Can you work these out from the model? Positions are in its coordinate system, mm. Coordinates: 2 decimals unless noted, no trailing zeros. Loops run counter-clockwise (first coordinate to the right, second up) from the corner with the lowest first, then second, coordinate; pieces in that order, holes last.
```python
from build123d import *

# Parameters (mm, degrees)
G1_1_4_TAPPED_HOLE1_D = 39.25
CHAMFER1_SIZE         = 1


with BuildPart() as part:
    # Sketch1 → Revolve1 (revolve)
    with BuildSketch(Plane(origin=(0, 0, 0), x_dir=(0, 0, -1), z_dir=(1, 0, 0)), mode=Mode.PRIVATE) as revolve1_sk:
        Polygon((0, 0), (0, 25), (-10, 25), (-10, 30), (-20, 30), (-20, 0), align=None)
    revolve(revolve1_sk.sketch.rotate(Axis((0, 0, 20), (0, 0, -1)), 90), axis=Axis((0, 0, 20), (0, 0, -1)))

    # G1-1/4 Tapped Hole1 (through all)
    with Locations(Plane.XY.offset(20)):
        with Locations((0, 0)):
            Hole(G1_1_4_TAPPED_HOLE1_D / 2)

    # Chamfer1
    chamfer1_edges = [part.edges().sort_by_distance(p)[0] for p in [
        (-30, 0, 20),
    ]]
    chamfer(chamfer1_edges, length=CHAMFER1_SIZE)


solid = part.part
```
(1) I want a section at A-A on x = 0. Write out the boundary of the cut face in (y, z) (3 decimals), then the cut area to 3 significant figures.
Check values:
outline: (-30, 10) - (-25, 10) - (-25, 0) - (-19.625, 0) - (-19.625, 20) - (-29, 20) - (-30, 19) - close; (19.625, 0) - (25, 0) - (25, 10) - (30, 10) - (30, 19) - (29, 20) - (19.625, 20) - close
area: 314 mm2
(2) If we mould it in two halves opening along X, with no side actions, what happens to faces 1 (the cylindrical face through (23.846, -7.509, 5.07)), 2 (the flat face through (7, -25, 10)), 3 (the cylindrical face through (19.606, 0.863, 9.86))? For each: released by +X, released by -X, zero draft, split by the parting line, or undercut.
Check values:
face 1: split by the parting line
face 2: zero draft
face 3: undercut
(3) I want a section at C-C on z = 6.75. Write out the boundary of the cut face in (x, y) (3 decimals), then the cut area to 3 significant figures.
Check values:
outline: circle Ø50 at (0, 0); hole circle Ø39.25 at (0, 0)
area: 754 mm2
(4) I'm going to push flat-ended pins straight in: pin 1 (10 mm diameter, centred on x = -13.5, z = 10.5, fed in from +Y); pin 2 (3 mm diameter, centred on y = 10.5, z = 6, fed in from -X); pin 3 (5 mm diameter, centred on x = 0, z = 13, fed in from -Y); pin 4 (23.5 mm diameter, centred on x = 0, y = 0, fed in from -Z). Where does each tip first touch, or does it pass through?
Check values:
pin 1: stops at y = 28.77
pin 2: stops at x = -23.32
pin 3: stops at y = -30
pin 4: passes through
(5) If I drill on probe 1 along Y at (x, z) = (0, 9) (3 decimals); probe 2 along X at (y, z) = (16, 6); probe 3 along Z at (x, y) = (-25, 10), over which ranges is the centre line in solid material (lowest first)?
Check values:
probe 1: y = -25 to -19.625, 19.625 to 25
probe 2: x = -19.21 to -11.36, 11.36 to 19.21
probe 3: z = 10 to 20
